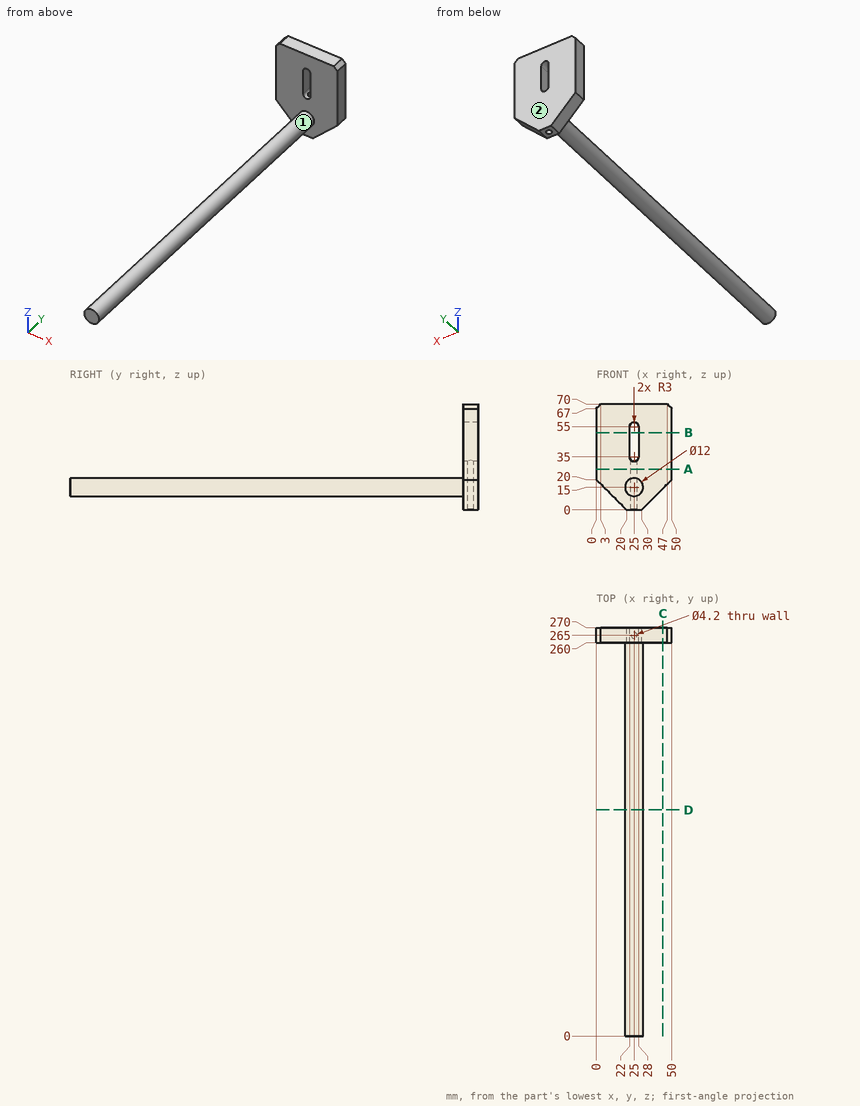
Geometry check sheet. Reference: drawing and pictorial views, mm from the part's lowest x, y, z. Coordinates: 2 decimals unless noted, no trailing zeros. Write each loop counter-clockwise with the first axis right and the second up, starting at its lowest first coordinate (ties: lowest second). Pieces come first, ordered by that corner, then holes. Notation, with made-up numbers: (-22.75, 8.5) -> (27.25, 8.5) arc R27 cw to (27.25, 29.5) -> close; hole circle Ø1 at (-25, 30). An arc over 180 degrees is marked (long way). One line per question, with ' | ' between items.
1. Cross-section at B-B on z = 51. Record the cut outline in (x, y), and give its area (3 significant figures).
Answers:
outline: (0, 260) -> (22, 260) -> (22, 270) -> (0, 270) -> close; (28, 260) -> (50, 260) -> (50, 270) -> (28, 270) -> close | area: 440 mm²
2. Thickness scan on probe 1 along Y at (x, z) = (25, 17); probe 2 along X at (y, z) = (265, 26); probe 3 along Y at (x, z) = (25, 22.5). Record the ranges inside material, lowest first. Write a range as from..to.
Answers:
probe 1: y = 0..262.9, 267.1..270 | probe 2: x = 0..22.9, 27.1..50 | probe 3: y = 260..262.9, 267.1..270
3. Cross-section at D-D on y = 149.5. Record the cut outline in (x, z).
Answers:
outline: circle Ø12 at (25, 15)
4. Cross-section at C-C on x = 44. Record the cut outline in (y, z), and give its area (3 significant figures).
Answers:
outline: (260, 14) -> (270, 14) -> (270, 70) -> (260, 70) -> close | area: 560 mm²
5. Depth check by flat-ended pin: pin 1 Ø1 at (x, z) = (15, 44.5) entering from -Y; pin 2 Ø3 at (y, z) = (267, 41.5) entering from -X; pin 3 Ø8 at (x, y) = (17, 237.5) entering from -Z. Enter the tip coordinate at first touch or a pass-through.
Answers:
pin 1: stops at y = 260 | pin 2: stops at x = 0 | pin 3: stops at z = 10.53
6. Draft check along Z on the marked faces 1 and 2. Enter one of: +Z half, -Z half, draft (parallel to the pull), parting line (faces both ways), or undercut.
Answers:
face 1: parting line | face 2: draft
7. Cross-section at A-A on z = 27. Record the cut outline in (x, y).
Answers:
outline: (0, 260) -> (50, 260) -> (50, 270) -> (0, 270) -> close; hole circle Ø4.2 at (25, 265)
